Could you check a few things on this model? Use its own coordinates, in mm. A direction names the side the tool comes from. Give positions to 0.01 mm unless a question says otherwise; leave off trailing zeros. Loops run counter-clockwise (first coordinate to the right, second up) from the corner with the lowest first, then second, coordinate; pieces in that order, holes last. Notation, with made-up numbers: M 46,-32 L 85,-32 A12 cw 85,-15 Z; hole C 33.25,-27 d7. An arc over 180 degrees is marked long. Write each question's results on one line, items separated by ' | '. Start each with the question number.
from build123d import *

# Parameters (mm, degrees)
EXTRUDE_5_DEPTH     = 7.5
SKETCH_7_W          = 40
SKETCH_7_H          = 30
EXTRUDE_6_DEPTH     = 12
SKETCH_8_W          = 30
SKETCH_8_H          = 30
CUT_EXTRUDE_1_DEPTH = 1.5


with BuildPart() as part:
    # 草图6 → 凸台-拉伸5 (new, symmetric)
    with BuildSketch(Plane.XY):
        Polygon((0, 0), (162, 0), (162, -25), (250, -25), (250, -37), (150, -37), (150, -12), (0, -12), align=None)
    extrude(amount=EXTRUDE_5_DEPTH, both=True)

    # 草图7 → 凸台-拉伸6 (add)
    with BuildSketch(Plane(origin=(0, 0, 0), x_dir=(1, 0, 0), z_dir=(0, 1, 0))):
        with Locations((-20, 0)):
            Rectangle(SKETCH_7_W, SKETCH_7_H)
    extrude(amount=-EXTRUDE_6_DEPTH)

    # 草图8 → 切除-拉伸1 (cut)
    with BuildSketch(Plane(origin=(0, -12, 0), x_dir=(1, 0, 0), z_dir=(0, 1, 0))):
        with Locations((-22, 0)):
            Rectangle(SKETCH_8_W, SKETCH_8_H)
    extrude(amount=CUT_EXTRUDE_1_DEPTH, mode=Mode.SUBTRACT)


solid = part.part
1) If we section it at D-D on z = 10.75: Write out the boundary of the cut face in (x, y), plus the area to 3 significant figures.
2) If we section it at C-C on y = -21.5: Write out the boundary of the cut face in (x, z).
3) Please list where these lines run through material, in increasing order: line 1 (X direction, y = -3.5, z = -9); line 2 (X direction, y = -28, z = -4.25); line 3 (Y direction, x = 11.5, z = 5). Write a range as from..to.
4) Which directions (+Z, -Z, +X, -X, +Y, -Y) give clear straight access to the entire face, cutting with the end or side of a thin tool? Please do faces 4 (the face through (-20, -6, 15)), 5 (the face through (162, -12, 0)), 6 (the face through (70, -12, 0)), 7 (the face through (127, -10, -7.5)), 8 (the face through (-20, -6, -15)).
5) If we section it at A-A on z = -4.5: Write out the boundary of the cut face in (x, y), plus the area to 4 significant figures.
6) If we section it at B-B on x = 39.5: Write out the boundary of the cut face in (y, z).
7) I'm going to push flat-ended pins straight in: P1, Ø3.5, axis at x = -38.5, z = 0.5, coming from the -Y side; P2, Ø1.2, axis at y = -11.5, z = 7, coming from the +X side; P3, Ø1, axis at y = -29, z = -2.5, coming from the -X side. Where does each tip first touch, or does it pass through?
8) Thinking about a two-plate mould opening in X: for faces 1 (the face through (0, -6, 11)), 2 (the face through (127, -10, 7.5)), 3 (the face through (-22, -10.5, 0)), which applies, pulls with the +X half, pulls with the -X half, needs draft (parallel to the pull), parting line crosses it, or undercut?
Calculated:
1) outline: M -40,-12 L -37,-12 L -37,-10.5 L -7,-10.5 L -7,-12 L 0,-12 L 0,0 L -40,0 Z | area: 435 mm2
2) outline: M 150,-7.5 L 162,-7.5 L 162,7.5 L 150,7.5 Z
3) line 1: x = -40..0 | line 2: x = 150..250 | line 3: y = -12..0
4) face 4: +Z, +X, -X, +Y, -Y | face 5: +Z, -Z, +X, +Y | face 6: +Z, -Z, -X, -Y | face 7: -Z, +X, +Y, -Y | face 8: -Z, +X, -X, +Y, -Y
5) outline: M -40,-12 L -37,-12 L -37,-10.5 L -7,-10.5 L -7,-12 L 150,-12 L 150,-37 L 250,-37 L 250,-25 L 162,-25 L 162,0 L -40,0 Z | area: 3,735 mm2
6) outline: M -12,-7.5 L 0,-7.5 L 0,7.5 L -12,7.5 Z
7) P1: stops at y = -12 | P2: stops at x = 162 | P3: stops at x = 150
8) face 1: pulls with the +X half | face 2: needs draft | face 3: undercut
